from build123d import *

# Parameters (mm, degrees)
EXTRUDE_1_DEPTH     = 615
SKETCH_2_W          = 18
SKETCH_2_H          = 6
CUT_EXTRUDE_1_DEPTH = 617.8062905
HOLE_WIZARD_M5_1_D  = 4.2


with BuildPart() as part:
    # 草图1 → 拉伸-薄壁1 (new, symmetric)
    with BuildSketch(Plane.XY):
        with BuildLine():
            Line((25, -20), (-22, -20))
            ThreePointArc((-22, -20), (-24.121320344, -19.121320344), (-25, -17))
            Line((-25, -17), (-25, 17))
            ThreePointArc((-25, 17), (-24.121320344, 19.121320344), (-22, 20))
            Line((-22, 20), (25, 20))
            Line((25, 20), (25, 18))
            Line((25, 18), (-22, 18))
            ThreePointArc((-22, 18), (-22.707106781, 17.707106781), (-23, 17))
            Line((-23, 17), (-23, -17))
            ThreePointArc((-23, -17), (-22.707106781, -17.707106781), (-22, -18))
            Line((-22, -18), (25, -18))
            Line((25, -18), (25, -20))
        make_face()
    extrude(amount=EXTRUDE_1_DEPTH, both=True)

    # 草图2 → 切除-拉伸1 (cut, through all)
    with BuildSketch(Plane.XZ.offset(20)):
        with Locations((25, 45)):
            Rectangle(SKETCH_2_W, SKETCH_2_H)
    extrude(amount=-CUT_EXTRUDE_1_DEPTH, mode=Mode.SUBTRACT)

    # M5 螺纹孔1 (through all)
    with Locations(Plane.ZY.offset(25)):
        with Locations((590, 0), (320, 0), (-320, 0), (-590, 0), (565.5, 0), (599, 0), (-599, 0), (-565.5, 0)):
            Hole(HOLE_WIZARD_M5_1_D / 2)


solid = part.part
Design review of the part built by this model. Coordinates are the model's own, in mm. A direction names the side the tool comes from. Round coordinates to 2 decimals unless told otherwise and drop trailing zeros. Loops run counter-clockwise (first coordinate to the right, second up) from the corner with the lowest first, then second, coordinate; pieces in that order, holes last. Notation, with made-up numbers: (78, -28.75) - (127, -28.75) arc R21 cw to (127, -3.75) - close; hole circle Ø5 at (-15.5, -33). An arc over 180 degrees is marked (long way). One line per item, written item: value. Start each with the question number.
1) Consider section B-B on z = -82. Give the boundary of the cut face in (x, y), then the cut area to 3 significant figures.
2) Insertion check: pin 1 Ø1.5 at (y, z) = (12, -2.5) entering from +X; pin 2 Ø1.6 at (y, z) = (19, 45) entering from +X. Each pin has a flat end and moves straight along its axis. Give the tip position at first contact, or say it passes through.
3) Consider section A-A on x = 0. Give the boundary of the cut face in (y, z), then the cut area to 3 significant figures.
4) Consider section C-C on y = 10. Give the boundary of the cut face in (x, z), then the cut area to 3 significant figures.
5) Draft analysis for pull direction Y (two halves, no side actions). For faces 1 (the flat face through (-25, 0, 9)), 2 (the flat face through (-23, 0, 9)), 3 (the flat face through (1, 20, 9)), 4 (the flat face through (2, -20, 9)), state which applies: +Y half, -Y half, draft (parallel to the pull), parting line (faces both ways), or undercut.
6) For faces 5 (the flat face through (-24, 0, 615)), 6 (the flat face through (2, 18, 9)), list the 3-axis set-ups (+Z, -Z, +X, -X, +Y, -Y) from which the entire face can be reached by the end or side of a thin tool; tool diameter is ignored.
7) To check wall thickness, follow L1, parallel to Y at x = 23, z = -218; L2, parallel to X at y = 3, z = 310.5; L3, parallel to Y at x = -24.3, z = 565.5. State the ranges of each line that lie inside material, in increasing order. Write a range as from..to.
Reported:
1. outline: (-25, -17) arc R3 ccw to (-22, -20) - (25, -20) - (25, -18) - (-22, -18) arc R1 cw to (-23, -17) - (-23, 17) arc R1 cw to (-22, 18) - (25, 18) - (25, 20) - (-22, 20) arc R3 ccw to (-25, 17) - close
1. area: 269 mm^2
2. pin 1: stops at x = -23
2. pin 2: stops at x = 16
3. outline: (-20, -615) - (-18, -615) - (-18, 615) - (-20, 615) - close; (18, -615) - (20, -615) - (20, 615) - (18, 615) - close
3. area: 4,920 mm^2
4. outline: (-25, -615) - (-23, -615) - (-23, 615) - (-25, 615) - close
4. area: 2,460 mm^2
5. face 1: draft
5. face 2: undercut
5. face 3: +Y half
5. face 4: -Y half
6. face 5: +Z, +X, -X, +Y, -Y
6. face 6: +Z, -Z, +X
7. L1: y = -20..-18, 18..20
7. L2: x = -25..-23
7. L3: y = -18.93..-2.1, 2.1..18.93
